Here's how the part is built. I have some questions about the finished solid (model axes, mm). Round coordinates to 2 decimals unless told otherwise and drop trailing zeros. Loops run counter-clockwise (first coordinate to the right, second up) from the corner with the lowest first, then second, coordinate; pieces in that order, holes last. Notation, with made-up numbers: (51.25, -29.75) -> (64.25, -29.75) arc R10 ccw to (64.25, -24.75) -> close; hole circle Ø8 at (21.5, 79). An arc over 180 degrees is marked (long way). Use one line per item in the form item = value. Start each with the question number.
Item 1: If we section it at D-D (x = 12.75): State how many separate pieces and enclosed holes the cut face has, then the cut area to 3 significant figures.
Item 2: I'm going to push flat-ended pins straight in: pin 1 Ø3.5 at (y, z) = (13, 53) entering from -X; pin 2 Ø5.5 at (y, z) = (13, 11.5) entering from +X; pin 3 Ø3 at (y, z) = (0.5, -49.5) entering from +X (1 decimal); pin 4 Ø3.5 at (y, z) = (13, -27) entering from +X. Where does each tip first touch, or does it pass through?
Item 3: If we section it at A-A (z = -49.5): Write out the boundary of the cut face in (x, y), then the cut area to 3 significant figures.
Item 4: If I drill on L1, parallel to Y at x = 10.75, z = -49.5; L2, parallel to Z at x = 12.5, y = 13; L3, parallel to Z at x = 10, y = -12.5, over which ranges is the centre line in solid material (lowest first)? Write a range as [from, to].
Item 5: If we section it at B-B (z = 33): Write out the boundary of the cut face in (x, y) (3 decimals).
Item 6: If we section it at C-C (y = 0.5): Write out the boundary of the cut face in (x, z).
```python
from build123d import *

# Parameters (mm, degrees)
SKETCH1_W                                            = 121
SKETCH1_H                                            = 40
BOSS_EXTRUDE1_DEPTH                                  = 15
M5_TAPPED_HOLE1_D                                    = 4.2
M5_TAPPED_HOLE1_DEPTH                                = 12.4
M5_TAPPED_HOLE1_TIP                                  = 1.2618073
M6_TAPPED_HOLE1_D                                    = 5
M6_TAPPED_HOLE1_DEPTH                                = 15
M6_TAPPED_HOLE1_CSINK_D                              = 6.05
M6_TAPPED_HOLE1_CSINK_ANGLE                          = 90
M6_TAPPED_HOLE1_TIP                                  = 1.502151548
CBORE_FOR_M6_HEXAGON_SOCKET_HEAD_CAP_SCR_D           = 6.6
CBORE_FOR_M6_HEXAGON_SOCKET_HEAD_CAP_SCR_CBORE_D     = 11
CBORE_FOR_M6_HEXAGON_SOCKET_HEAD_CAP_SCR_CBORE_DEPTH = 6.8
F_5_0MM_BLIND_HOLE_1_D                               = 5
F_5_0MM_BLIND_HOLE_1_CSINK_D                         = 5.4
F_5_0MM_BLIND_HOLE_1_CSINK_ANGLE                     = 90
CHAMFER1_SIZE                                        = 3


with BuildPart() as part:
    # Sketch1 → Boss-Extrude1 (new body)
    with BuildSketch(Plane(origin=(0, 0, 0), x_dir=(0, 0, -1), z_dir=(1, 0, 0))):
        Rectangle(SKETCH1_W, SKETCH1_H)
    extrude(amount=BOSS_EXTRUDE1_DEPTH)

    # M5 Tapped Hole1
    with Locations(Plane(origin=(15, 0, 0), x_dir=(0, 0, -1), z_dir=(1, 0, 0))):
        with Locations((-53, 13), (27, 13)):
            Hole(M5_TAPPED_HOLE1_D / 2, depth=M5_TAPPED_HOLE1_DEPTH)
            with Locations((0, 0, -(M5_TAPPED_HOLE1_DEPTH + M5_TAPPED_HOLE1_TIP / 2))):  # 118° drill point
                Cone(0, M5_TAPPED_HOLE1_D / 2, M5_TAPPED_HOLE1_TIP, mode=Mode.SUBTRACT)

    # M6 Tapped Hole1
    with Locations(Plane(origin=(15, 0, 0), x_dir=(0, 0, -1), z_dir=(1, 0, 0))):
        with Locations((-33, -12.5), (7, -12.5)):
            CounterSinkHole(M6_TAPPED_HOLE1_D / 2, M6_TAPPED_HOLE1_CSINK_D / 2, depth=M6_TAPPED_HOLE1_DEPTH, counter_sink_angle=M6_TAPPED_HOLE1_CSINK_ANGLE)
            with Locations((0, 0, -(M6_TAPPED_HOLE1_DEPTH + M6_TAPPED_HOLE1_TIP / 2))):  # 118° drill point
                Cone(0, M6_TAPPED_HOLE1_D / 2, M6_TAPPED_HOLE1_TIP, mode=Mode.SUBTRACT)

    # CBORE for M6 Hexagon socket head cap screws1 (through all)
    with Locations(Plane(origin=(15, 0, 0), x_dir=(0, 0, -1), z_dir=(1, 0, 0))):
        with Locations((-10.5, 12.5), (49.5, 12.5)):
            CounterBoreHole(CBORE_FOR_M6_HEXAGON_SOCKET_HEAD_CAP_SCR_D / 2, CBORE_FOR_M6_HEXAGON_SOCKET_HEAD_CAP_SCR_CBORE_D / 2, CBORE_FOR_M6_HEXAGON_SOCKET_HEAD_CAP_SCR_CBORE_DEPTH)

    # Ø5.0mm blind hole 1 (through all)
    with Locations(Plane(origin=(15, 0, 0), x_dir=(0, 0, -1), z_dir=(1, 0, 0))):
        with Locations((-10.5, 0.5), (49.5, 0.5)):
            CounterSinkHole(F_5_0MM_BLIND_HOLE_1_D / 2, F_5_0MM_BLIND_HOLE_1_CSINK_D / 2, counter_sink_angle=F_5_0MM_BLIND_HOLE_1_CSINK_ANGLE)

    # Chamfer1
    chamfer1_edges = [part.edges().sort_by_distance(p)[0] for p in [
        (7.5, -20, -60.5),
        (7.5, -20, 60.5),
        (7.5, 20, 60.5),
        (7.5, 20, -60.5),
    ]]
    chamfer(chamfer1_edges, length=CHAMFER1_SIZE)


solid = part.part
```
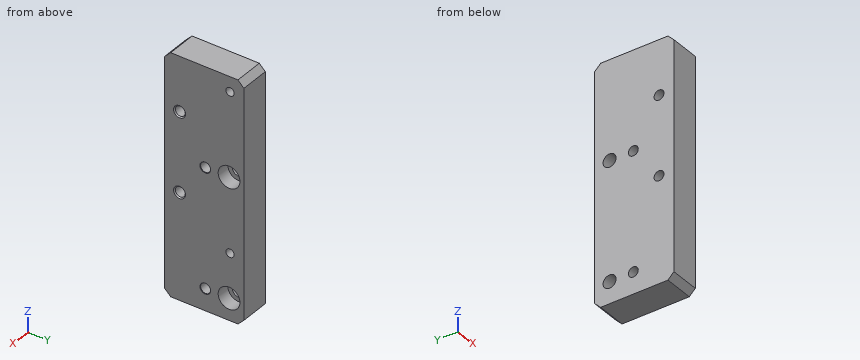
Values found:
q1.separate_pieces = 1
q1.enclosed_holes = 8
q1.area = 4,530 mm2
q2.pin_1 = 0
q2.pin_2 = 8.2
q2.pin_3 = through
q2.pin_4 = 2.39
q3.outline = (0, -20) -> (15, -20) -> (15, -2.2) -> (14.8, -2) -> (0, -2) -> close; (0, 3) -> (14.8, 3) -> (15, 3.2) -> (15, 7) -> (8.2, 7) -> (8.2, 9.2) -> (0, 9.2) -> close; (0, 15.8) -> (8.2, 15.8) -> (8.2, 18) -> (15, 18) -> (15, 20) -> (0, 20) -> close
q3.area = 396 mm2
q4.L1 = [-20, -2], [3, 7], [18, 20]
q4.L2 = [-60.5, -54.98], [-44.02, -29.1], [-24.9, 5.02], [15.98, 50.9], [55.1, 60.5]
q4.L3 = [-60.5, -9.5], [-4.5, 30.5], [35.5, 60.5]
q5.outline = (0, -20) -> (15, -20) -> (15, -15.525) -> (14.475, -15) -> (0, -15) -> close; (0, -10) -> (14.475, -10) -> (15, -9.475) -> (15, 20) -> (0, 20) -> close
q6.outline = (0, -60.5) -> (15, -60.5) -> (15, -52.2) -> (14.8, -52) -> (0, -52) -> close; (0, -47) -> (14.8, -47) -> (15, -46.8) -> (15, 7.8) -> (14.8, 8) -> (0, 8) -> close; (0, 13) -> (14.8, 13) -> (15, 13.2) -> (15, 60.5) -> (0, 60.5) -> close
